Can you work these out from the drawing? Everything is in mm from the part's minimum corner. Coordinates: 2 decimals unless noted, no trailing zeros. Loops run counter-clockwise (first coordinate to the right, second up) from the corner with the lowest first, then second, coordinate; pieces in that order, holes last.
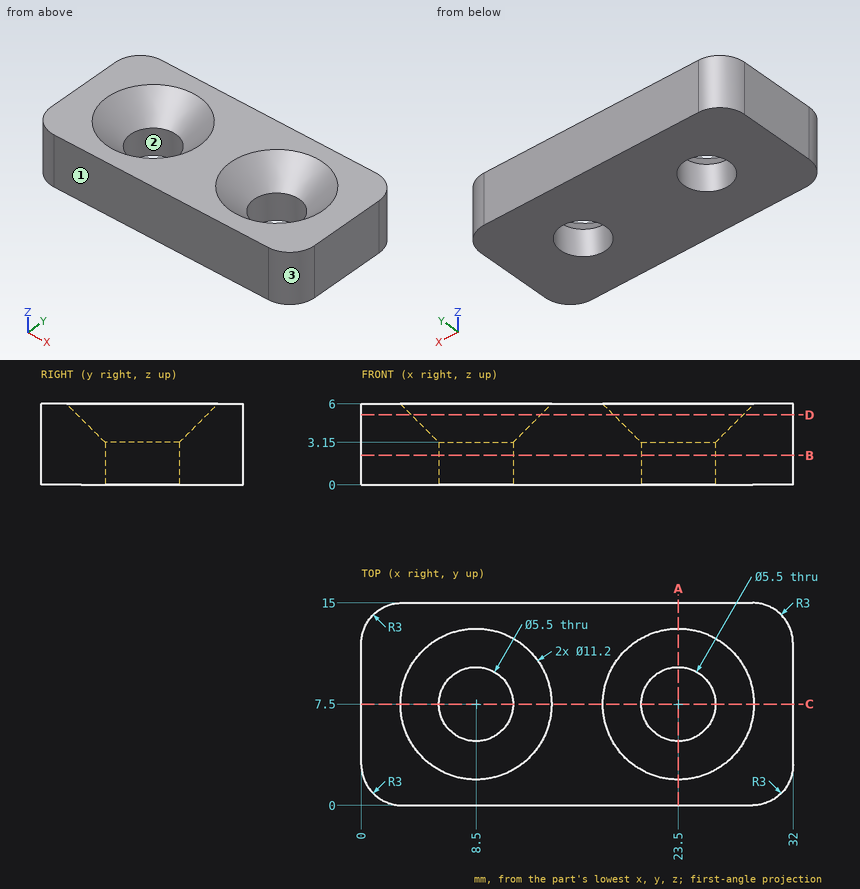
1. I want a section at B-B (z = 2.2). Please give me the cut outline in (x, y), then the cut area to 3 significant figures.
2. I want a section at C-C (y = 7.5). Please give me the cut outline in (x, z), then the cut area to 3 significant figures.
3. We'd pull the mould along X, two halves only. Please class the marked faces 1, 2 and 3: +X half, -X half, draft (parallel to the pull), parting line (faces both ways), or undercut.
4. I want a section at A-A (x = 23.5). Please give me the cut outline in (y, z), then the cut area to 3 significant figures.
5. I need wall thicknesses on line 1 along X through (y, z) = (7.5, 2.3); line 2 along Y through (x, z) = (8.5, 0.6); line 3 along X through (y, z) = (6.5, 5.3). Which ranges of each line are inside material? Lowest first, please.
6. I want a section at D-D (z = 5.2). Please give me the cut outline in (x, y).
Response values:
1. outline: (0, 3) arc R3 ccw to (3, 0) - (29, 0) arc R3 ccw to (32, 3) - (32, 12) arc R3 ccw to (29, 15) - (3, 15) arc R3 ccw to (0, 12) - close; hole circle Ø5.5 at (8.5, 7.5); hole circle Ø5.5 at (23.5, 7.5)
1. area: 425 mm2
2. outline: (0, 0) - (5.75, 0) - (5.75, 3.15) - (2.9, 6) - (0, 6) - close; (11.25, 0) - (20.75, 0) - (20.75, 3.15) - (17.9, 6) - (14.1, 6) - (11.25, 3.15) - close; (26.25, 0) - (32, 0) - (32, 6) - (29.1, 6) - (26.25, 3.15) - close
2. area: 110 mm2
3. face 1: draft
3. face 2: undercut
3. face 3: +X half
4. outline: (0, 0) - (4.75, 0) - (4.75, 3.15) - (1.9, 6) - (0, 6) - close; (10.25, 0) - (15, 0) - (15, 6) - (13.1, 6) - (10.25, 3.15) - close
4. area: 48.9 mm2
5. line 1: x = 0 to 5.75, 11.25 to 20.75, 26.25 to 32
5. line 2: y = 0 to 4.75, 10.25 to 15
5. line 3: x = 0 to 3.7, 13.3 to 18.7, 28.3 to 32
6. outline: (0, 3) arc R3 ccw to (3, 0) - (29, 0) arc R3 ccw to (32, 3) - (32, 12) arc R3 ccw to (29, 15) - (3, 15) arc R3 ccw to (0, 12) - close; hole circle Ø9.6 at (8.5, 7.5); hole circle Ø9.6 at (23.5, 7.5)
